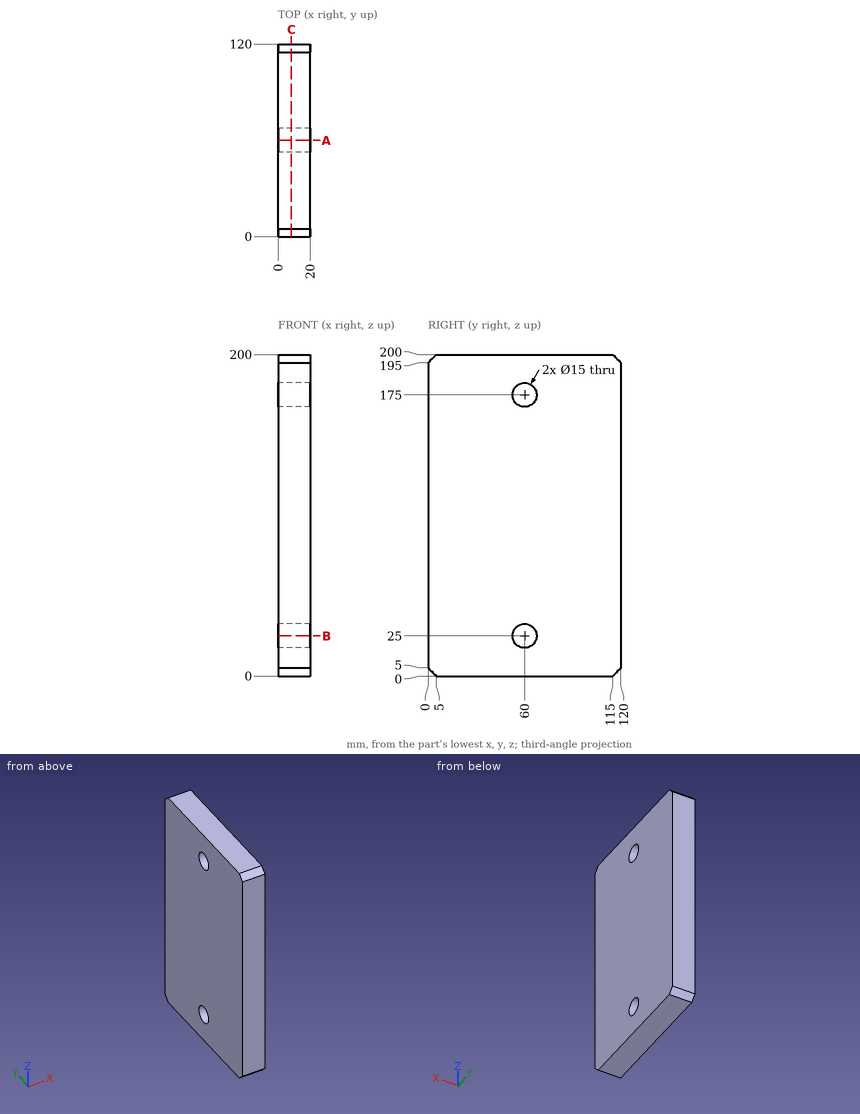
Answer from the drawing. Dimensions are ordinates in mm from the lowest x, y and z of the part. Give positions to 0.01 mm unless a question says otherwise; leave off trailing zeros. Order: outer loops, then holes, each group sorted by start corner. A loop starts at its lowest first (then second) coordinate and runs counter-clockwise, first axis right, second up. Notation, with made-up numbers: (22.5, 85.5) - (58.5, 85.5) arc R24 cw to (58.5, 123.5) - close; hole circle Ø9 at (67, 84). An arc over 180 degrees is marked (long way). One line per item, written item: value. Start each with the question number.
1) Find the intervals of material crossed by L1, parallel to Z at x = 14, y = 65.5; L2, parallel to Y at x = 14, z = 25; L3, parallel to Y at x = 8.25, z = 170, in increasing order.
2) A cutting plane is placed at B-B on z = 25. Give the vertices of the cut face in (x, y).
3) A cutting plane is placed at C-C on x = 8.25. Give the vertices of the cut face in (y, z), then the cut area to 3 significant figures.
4) Given pin 1 Ø12 at (x, y) = (2, 54) entering from -Z; pin 2 Ø13.5 at (y, z) = (60, 25) entering from -X, each flat-ended and moving along its own axis, determine where each tip first touches the part or whether it passes through.
5) A cutting plane is placed at A-A on y = 60. Give the vertices of the cut face in (x, z), then the cut area to 3 significant figures.
Answer sheet:
1. L1: z = 0 to 19.9, 30.1 to 169.9, 180.1 to 200
1. L2: y = 0 to 52.5, 67.5 to 120
1. L3: y = 0 to 54.41, 65.59 to 120
2. outline: (0, 0) - (20, 0) - (20, 52.5) - (0, 52.5) - close; (0, 67.5) - (20, 67.5) - (20, 120) - (0, 120) - close
3. outline: (0, 5) - (5, 0) - (115, 0) - (120, 5) - (120, 195) - (115, 200) - (5, 200) - (0, 195) - close; hole circle Ø15 at (60, 25); hole circle Ø15 at (60, 175)
3. area: 23,600 mm2
4. pin 1: stops at z = 0
4. pin 2: passes through
5. outline: (0, 0) - (20, 0) - (20, 17.5) - (0, 17.5) - close; (0, 32.5) - (20, 32.5) - (20, 167.5) - (0, 167.5) - close; (0, 182.5) - (20, 182.5) - (20, 200) - (0, 200) - close
5. area: 3,400 mm2
